```python
from build123d import *

# Parameters (mm, degrees)
CHAMFER1_SIZE      = 0.35
CUT_EXTRUDE1_START = -1.3
CUT_EXTRUDE1_DEPTH = 1.3


with BuildPart() as part:
    # Sketch1 → Base-Revolve (revolve)
    with BuildSketch(Plane.XY, mode=Mode.PRIVATE) as base_revolve_sk:
        with BuildLine():
            Line((0, 0), (0, 4.2))
            Line((0, 4.2), (0.1969, 4.2))
            Line((0.1969, 4.2), (2.407106781, 1.989793219))
            ThreePointArc((2.407106781, 1.989793219), (2.73153013, 1.773020467), (3.114213562, 1.6969))
            Line((3.114213562, 1.6969), (3.5750154, 1.6969))
            Line((3.5750154, 1.6969), (4.1, 2))
            Line((4.1, 2), (8, 2))
            Line((8, 2), (8, 0))
            Line((8, 0), (0, 0))
        make_face()
    revolve(base_revolve_sk.sketch.rotate(Axis((0, 0, 0), (1, 0, 0)), 90), axis=Axis((0, 0, 0), (1, 0, 0)))

    # Chamfer1
    chamfer1_edges = [part.edges().sort_by_distance(p)[0] for p in [
        (8, 0, -2),
    ]]
    chamfer(chamfer1_edges, length=CHAMFER1_SIZE)

    # Sketch3 → Cut-Extrude1 (cut)
    with BuildSketch(Plane.ZY.offset(CUT_EXTRUDE1_START)):
        with BuildLine():
            Line((-4.156921938, 0.6), (4.156921938, 0.6))
            ThreePointArc((4.156921938, 0.6), (4.2, 0), (4.156921938, -0.6))
            Line((4.156921938, -0.6), (-4.156921938, -0.6))
            ThreePointArc((-4.156921938, -0.6), (-4.2, 0), (-4.156921938, 0.6))
        make_face()
    extrude(amount=CUT_EXTRUDE1_DEPTH, mode=Mode.SUBTRACT)


solid = part.part
```
Could you check a few things on this model? Use its own coordinates, in mm. A direction names the side the tool comes from. Give positions to 0.01 mm unless a question says otherwise; leave off trailing zeros. Loops run counter-clockwise (first coordinate to the right, second up) from the corner with the lowest first, then second, coordinate; pieces in that order, holes last. Notation, with made-up numbers: (9, 84.25) -> (57, 84.25) arc R27 ccw to (57, 115.25) -> close; hole circle Ø1 at (82, 22). An arc over 180 degrees is marked (long way). Put each result on its own line as item: value.
(1) Imagine slicing it at B-B on z = 0. Write out the boundary of the cut face in (x, y), plus the area to 3 significant figures.
Computed:
outline: (0, -4.2) -> (0.2, -4.2) -> (2.41, -1.99) arc R1 cw to (3.11, -1.7) -> (3.58, -1.7) -> (4.1, -2) -> (7.65, -2) -> (8, -1.65) -> (8, 1.65) -> (7.65, 2) -> (4.1, 2) -> (3.58, 1.7) -> (3.11, 1.7) arc R1 cw to (2.41, 1.99) -> (0.2, 4.2) -> (0, 4.2) -> (0, 0.6) -> (1.3, 0.6) -> (1.3, -0.6) -> (0, -0.6) -> close
area: 35.3 mm^2
(2) Please list where these lines run through material, in increasing order: probe 1 along X at (y, z) = (-0.5, 0.5); probe 2 along X at (y, z) = (-0.75, -3); probe 3 along X at (y, z) = (-1.25, -1.25). Write a range as [from, to].
Computed:
probe 1: [1.3, 8]
probe 2: [0, 1.3]
probe 3: [0, 2.74], [3.7, 7.88]
(3) I'm going to push flat-ended pins straight in: pin 1 Ø1.5 at (y, z) = (-3, -3) entering from +X; pin 2 Ø2 at (x, y) = (6.5, 2.5) entering from +Z; pin 3 Ø3 at (x, z) = (2.5, 1) entering from -Y. Where does each tip first touch, or does it pass through?
Computed:
pin 1: x = 0.9
pin 2: z = 1.32
pin 3: y = -3.29
(4) For faces 1 (the face through (0, -2, 0)), 2 (the face through (1.3, 0, 0)), 3 (the face through (6, 2, 0)), which set-ups out of +Z, -Z, +X, -X, +Y, -Y let a thin tool reach every point of the face, with its end or its side?
Computed:
face 1: +Z, -Z, -X, +Y, -Y
face 2: +Z, -Z, -X
face 3: +X
(5) Imagine slicing it at D-D on x = 2.75. Write out the boundary of the cut face in (y, z).
Computed:
outline: circle Ø3.53 at (0, 0)
(6) Imagine slicing it at C-C on x = 6.75. Write out the boundary of the cut face in (y, z).
Computed:
outline: circle Ø4 at (0, 0)
(7) Thinking about a two-plate mould opening in X: for faces 4 (the face through (1, -0.6, 0)), 5 (the face through (0, 2, 0)), 6 (the face through (3.348, 1.657, -0.368)), 7 (the face through (8, 0, 0)), which applies, pulls with the +X half, pulls with the -X half, needs draft (parallel to the pull), parting line crosses it, or undercut?
Computed:
face 4: needs draft
face 5: pulls with the -X half
face 6: undercut
face 7: pulls with the +X half
(8) Imagine slicing it at A-A on y = 0. Write out the boundary of the cut face in (x, z).
Computed:
outline: (1.3, -3.1) -> (2.41, -1.99) arc R1 cw to (3.11, -1.7) -> (3.58, -1.7) -> (4.1, -2) -> (7.65, -2) -> (8, -1.65) -> (8, 1.65) -> (7.65, 2) -> (4.1, 2) -> (3.58, 1.7) -> (3.11, 1.7) arc R1 cw to (2.41, 1.99) -> (1.3, 3.1) -> close
